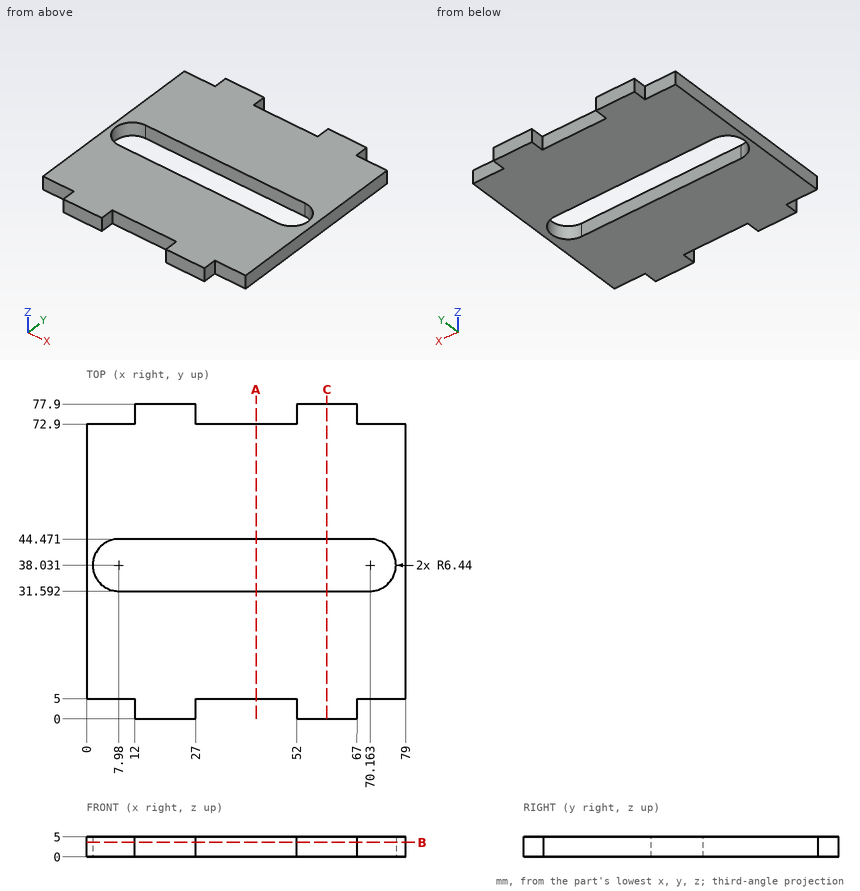
Verification items for this drawing (mm, ordinates from the low corner). Coordinates: 2 decimals unless noted, no trailing zeros. Loops run counter-clockwise (first coordinate to the right, second up) from the corner with the lowest first, then second, coordinate; pieces in that order, holes last.
Item 1: Go/stop test with flat-tipped pins: pin 1 Ø2.5 at (y, z) = (2, 1.5) entering from -X; pin 2 Ø1.5 at (x, z) = (8, 1) entering from +Y; pin 3 Ø2.5 at (x, z) = (73.5, 2) entering from -Y. Record where each tip stops, or that it passes through.
Item 2: Sectioned sample at A-A, the plane x = 42. Record the boundary of the cut face in (y, z), then the cut area to 3 significant figures.
Item 3: Thickness scan on line 1 (Y direction, x = 58, z = 2.2); line 2 (Y direction, x = 32.5, z = 0.7). Record the ranges inside material, lowest first.
Item 4: Sectioned sample at C-C, the plane x = 59.5. Record the boundary of the cut face in (y, z), then the cut area to 3 significant figures.
Item 5: Sectioned sample at B-B, the plane z = 3.6. Record the boundary of the cut face in (x, y).
Check result:
1. pin 1: stops at x = 12
1. pin 2: stops at y = 72.9
1. pin 3: stops at y = 5
2. outline: (5, 0) - (31.59, 0) - (31.59, 5) - (5, 5) - close; (44.47, 0) - (72.9, 0) - (72.9, 5) - (44.47, 5) - close
2. area: 275 mm2
3. line 1: y = 0 to 31.59, 44.47 to 77.9
3. line 2: y = 5 to 31.59, 44.47 to 72.9
4. outline: (0, 0) - (31.59, 0) - (31.59, 5) - (0, 5) - close; (44.47, 0) - (77.9, 0) - (77.9, 5) - (44.47, 5) - close
4. area: 325 mm2
5. outline: (0, 5) - (12, 5) - (12, 0) - (27, 0) - (27, 5) - (52, 5) - (52, 0) - (67, 0) - (67, 5) - (79, 5) - (79, 72.9) - (67, 72.9) - (67, 77.9) - (52, 77.9) - (52, 72.9) - (27, 72.9) - (27, 77.9) - (12, 77.9) - (12, 72.9) - (0, 72.9) - close; hole (7.98, 31.59) - (70.16, 31.59) arc R6.44 ccw to (70.16, 44.47) - (7.98, 44.47) arc R6.44 ccw to start
